Job drawing, mm, ordinate dimensions from the low corner. One solid piece. Give positions to 0.01 mm unless a question says otherwise; leave off trailing zeros. Write each loop counter-clockwise with the first axis right and the second up, starting at its lowest first coordinate (ties: lowest second). Pieces come first, ordered by that corner, then holes. Notation, with made-up numbers: (47, 20.5) - (101, 20.5) arc R17 cw to (101, 30.5) - close; hole circle Ø6 at (10.25, -34.5). An arc over 180 degrees is marked (long way). Answer as a JSON object with one key per item and string values.
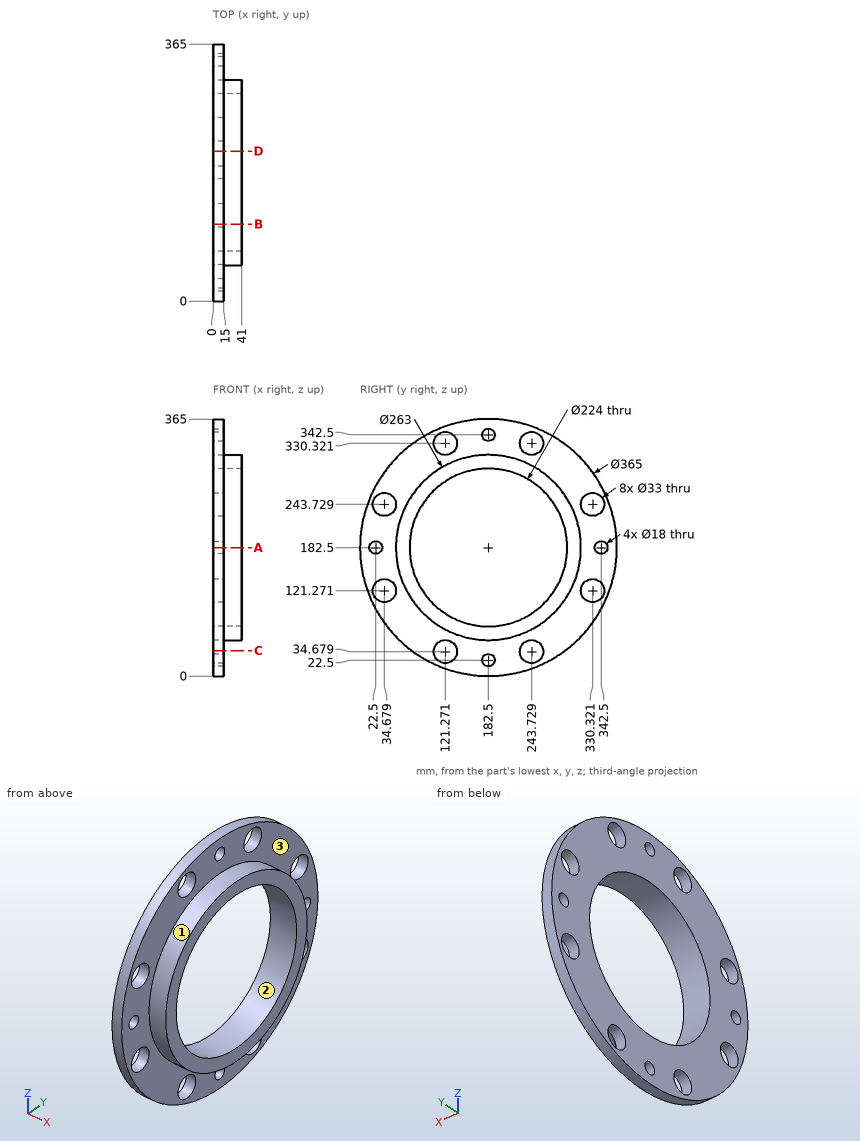
Item 1: Cut at B-B (y = 109). Give the cut face in (x, z) (1 decimal), and give its area (3 significant figures).
Entries:
{"outline": "(0, 15.5) - (15, 15.5) - (15, 23.6) - (0, 23.6) - close; (0, 45.7) - (15, 45.7) - (15, 73.5) - (41, 73.5) - (41, 98) - (0, 98) - close; (0, 267) - (41, 267) - (41, 291.5) - (15, 291.5) - (15, 319.3) - (0, 319.3) - close; (0, 341.4) - (15, 341.4) - (15, 349.5) - (0, 349.5) - close", "area": "3,090 mm2"}
Item 2: Cut at C-C (z = 36). Give the cut face in (x, y), and give its area (3 significant figures).
Entries:
{"outline": "(0, 73.67) - (15, 73.67) - (15, 104.82) - (0, 104.82) - close; (0, 137.72) - (15, 137.72) - (15, 227.28) - (0, 227.28) - close; (0, 260.18) - (15, 260.18) - (15, 291.33) - (0, 291.33) - close", "area": "2,280 mm2"}
Item 3: Flat gauge pins, fed straight in: P1, Ø6, axis at x = 24, z = 150, coming from the -Y side; P2, Ø2, axis at x = 29.5, z = 109, coming from the -Y side; P3, Ø2, axis at y = 75, z = 58.5, coming from the +X side; P4, Ø20, axis at y = 330.32, z = 121.27, coming from the -X side. Where does each tip first touch, or does it go through?
Entries:
{"P1": "y = 54.35", "P2": "y = 72.79", "P3": "x = 15", "P4": "through"}
Item 4: Probe line 1 (Y direction, x = 9, z = 182); line 2 (Y direction, x = 9, z = 255.5) (1 decimal). List the from-to ranges inside material, lowest first. Write a range as from..to.
Entries:
{"line 1": "0..13.51, 31.49..70.5, 294.5..333.51, 351.49..365", "line 2": "15.2..23.1, 46.2..97.6, 267.4..318.8, 341.9..349.8"}
Item 5: Mould opens along Y. For the marked faces 1, 2 and 3 say: +Y half, -Y half, draft (parallel to the pull), parting line (faces both ways), or undercut.
Entries:
{"face 1": "parting line", "face 2": "undercut", "face 3": "draft"}
Item 6: Cut at D-D (y = 213). Give the cut face in (x, z), and give its area (3 significant figures).
Entries:
{"outline": "(0, 2.57) - (15, 2.57) - (15, 54.59) - (41, 54.59) - (41, 74.73) - (0, 74.73) - close; (0, 290.27) - (41, 290.27) - (41, 310.41) - (15, 310.41) - (15, 362.43) - (0, 362.43) - close", "area": "3,210 mm2"}
Item 7: Cut at A-A (z = 182.5). Give the cut face in (x, y), and give its area (3 significant figures).
Entries:
{"outline": "(0, 0) - (15, 0) - (15, 13.5) - (0, 13.5) - close; (0, 31.5) - (15, 31.5) - (15, 51) - (41, 51) - (41, 70.5) - (0, 70.5) - close; (0, 294.5) - (41, 294.5) - (41, 314) - (15, 314) - (15, 333.5) - (0, 333.5) - close; (0, 351.5) - (15, 351.5) - (15, 365) - (0, 365) - close", "area": "2,590 mm2"}
